The model under review builds one solid part; all positions refer to its coordinate system, in mm. A direction names the side the tool comes from. Round coordinates to 2 decimals unless told otherwise and drop trailing zeros. Loops run counter-clockwise (first coordinate to the right, second up) from the corner with the lowest first, then second, coordinate; pieces in that order, holes last. Notation, with made-up numbers: M 52,11.25 L 95,11.25 A15 ccw 95,24.25 Z; hole C 25.25,64.5 d3. An arc over 180 degrees is marked long. One line per question, with ' | ' between items.
from build123d import *

# Parameters (mm, degrees)
SKETCH1_W                                          = 80
SKETCH1_H                                          = 100
BOSS_EXTRUDE1_DEPTH                                = 120
SKETCH2_R                                          = 20
CUT_EXTRUDE1_DEPTH                                 = 137.014705087
HOLE_SIZE_BASED_ON_HEX_SOCKET_CAP_SCRE_D           = 10
HOLE_SIZE_BASED_ON_HEX_SOCKET_CAP_SCRE_DEPTH       = 35
HOLE_SIZE_BASED_ON_HEX_SOCKET_CAP_SCRE_CBORE_D     = 15
HOLE_SIZE_BASED_ON_HEX_SOCKET_CAP_SCRE_CBORE_DEPTH = 9
HOLE_SIZE_BASED_ON_HEX_SOCKET_CAP_SCRE_TIP         = 3.004303095
HOLE_WIZARD_2_D                                    = 10
HOLE_WIZARD_2_DEPTH                                = 50
HOLE_WIZARD_2_CBORE_D                              = 15
HOLE_WIZARD_2_CBORE_DEPTH                          = 9
HOLE_WIZARD_2_TIP                                  = 3.004303095
M8_TAPPED_HOLE1_D                                  = 6.8
M8_TAPPED_HOLE1_DEPTH                              = 30
M8_TAPPED_HOLE1_TIP                                = 2.042926105
M8_TAPPED_HOLE2_D                                  = 6.8
M8_TAPPED_HOLE2_DEPTH                              = 30
M8_TAPPED_HOLE2_TIP                                = 2.042926105
M8_TAPPED_HOLE3_D                                  = 6.8
M8_TAPPED_HOLE3_DEPTH                              = 45
M8_TAPPED_HOLE3_TIP                                = 2.042926105


with BuildPart() as part:
    # Sketch1 → Boss-Extrude1 (new body)
    with BuildSketch(Plane.XY):
        Rectangle(SKETCH1_W, SKETCH1_H)
    extrude(amount=BOSS_EXTRUDE1_DEPTH)

    # Sketch2 → Cut-Extrude1 (cut, through all)
    with BuildSketch(Plane.XY.offset(120)):
        Circle(SKETCH2_R)
    extrude(amount=-CUT_EXTRUDE1_DEPTH, mode=Mode.SUBTRACT)

    # Hole Size (based on) hex socket cap screw type 2
    with Locations(Plane(origin=(0, 50, 0), x_dir=(1, 0, 0), z_dir=(0, 1, 0))):
        with Locations((0, -20), (0, -100)):
            CounterBoreHole(HOLE_SIZE_BASED_ON_HEX_SOCKET_CAP_SCRE_D / 2, HOLE_SIZE_BASED_ON_HEX_SOCKET_CAP_SCRE_CBORE_D / 2, HOLE_SIZE_BASED_ON_HEX_SOCKET_CAP_SCRE_CBORE_DEPTH, depth=HOLE_SIZE_BASED_ON_HEX_SOCKET_CAP_SCRE_DEPTH)
            with Locations((0, 0, -(HOLE_SIZE_BASED_ON_HEX_SOCKET_CAP_SCRE_DEPTH + HOLE_SIZE_BASED_ON_HEX_SOCKET_CAP_SCRE_TIP / 2))):  # 118° drill point
                Cone(0, HOLE_SIZE_BASED_ON_HEX_SOCKET_CAP_SCRE_D / 2, HOLE_SIZE_BASED_ON_HEX_SOCKET_CAP_SCRE_TIP, mode=Mode.SUBTRACT)

    # 打孔尺寸(%根据)内六角圆柱头螺钉的类型2
    with Locations(Plane(origin=(0, -50, 0), x_dir=(-1, 0, 0), z_dir=(0, -1, 0))):
        with Locations((0, -20), (0, -100)):
            CounterBoreHole(HOLE_WIZARD_2_D / 2, HOLE_WIZARD_2_CBORE_D / 2, HOLE_WIZARD_2_CBORE_DEPTH, depth=HOLE_WIZARD_2_DEPTH)
            with Locations((0, 0, -(HOLE_WIZARD_2_DEPTH + HOLE_WIZARD_2_TIP / 2))):  # 118° drill point
                Cone(0, HOLE_WIZARD_2_D / 2, HOLE_WIZARD_2_TIP, mode=Mode.SUBTRACT)

    # M8 Tapped Hole1
    with Locations(Plane.ZY.offset(40)):
        with Locations((30, 30), (90, 30), (90, -30), (30, -30)):
            Hole(M8_TAPPED_HOLE1_D / 2, depth=M8_TAPPED_HOLE1_DEPTH)
            with Locations((0, 0, -(M8_TAPPED_HOLE1_DEPTH + M8_TAPPED_HOLE1_TIP / 2))):  # 118° drill point
                Cone(0, M8_TAPPED_HOLE1_D / 2, M8_TAPPED_HOLE1_TIP, mode=Mode.SUBTRACT)

    # M8 Tapped Hole2
    with Locations(Plane(origin=(40, 0, 0), x_dir=(0, 0, -1), z_dir=(1, 0, 0))):
        with Locations((-90, 30), (-30, 30), (-30, -30), (-90, -30)):
            Hole(M8_TAPPED_HOLE2_D / 2, depth=M8_TAPPED_HOLE2_DEPTH)
            with Locations((0, 0, -(M8_TAPPED_HOLE2_DEPTH + M8_TAPPED_HOLE2_TIP / 2))):  # 118° drill point
                Cone(0, M8_TAPPED_HOLE2_D / 2, M8_TAPPED_HOLE2_TIP, mode=Mode.SUBTRACT)

    # M8 Tapped Hole3
    with Locations(Plane(origin=(0, 50, 0), x_dir=(1, 0, 0), z_dir=(0, 1, 0))):
        with Locations((0, -60)):
            Hole(M8_TAPPED_HOLE3_D / 2, depth=M8_TAPPED_HOLE3_DEPTH)
            with Locations((0, 0, -(M8_TAPPED_HOLE3_DEPTH + M8_TAPPED_HOLE3_TIP / 2))):  # 118° drill point
                Cone(0, M8_TAPPED_HOLE3_D / 2, M8_TAPPED_HOLE3_TIP, mode=Mode.SUBTRACT)


solid = part.part
1) Mouldability with a two-part tool opening along Z and no side actions: class faces 1 (the flat face through (17, 12, 0)), 2 (the flat face through (5, 41, 22)), 3 (the cylindrical face through (1.08, 30.03, 24.88)), 4 (the flat face through (-40, -1, 59)) as +Z half, -Z half, draft (parallel to the pull), parting line (faces both ways), or undercut.
Output values:
face 1: -Z half | face 2: undercut | face 3: undercut | face 4: draft
2) Add section C-C on x = 16.5. State the section outline as (y, z) points, then the cut area to 3 significant figures.
Output values:
outline: M -50,0 L -11.3,0 L -11.3,120 L -50,120 Z; M 11.3,0 L 50,0 L 50,120 L 11.3,120 Z; hole C -30,30 d6.8; hole C -30,90 d6.8; hole C 30,30 d6.8; hole C 30,90 d6.8 | area: 9,140 mm²
3) Add section A-A on y = 43.5. State the section outline as (x, z) points, then the cut area to 3 significant figures.
Output values:
outline: M -40,0 L 40,0 L 40,120 L -40,120 Z; hole C 0,20 d15; hole C 0,100 d15; hole C 0,60 d6.8 | area: 9,210 mm²
4) For line 1 (Z direction, x = 0, y = -30); line 2 (Z direction, x = 0, y = 47.5); line 3 (Z direction, x = -25.75, y = -30), list the stretches that pass through material, from the lowest coordinate up.
Output values:
line 1: z = 0 to 15, 25 to 95, 105 to 120 | line 2: z = 0 to 12.5, 27.5 to 56.6, 63.4 to 92.5, 107.5 to 120 | line 3: z = 0 to 26.6, 33.4 to 86.6, 93.4 to 120
5) Add section B-B on z = 20. State the section outline as (x, y) points, then the cut area to 3 significant figures.
Output values:
outline: M -40,-50 L -7.5,-50 L -7.5,-41 L -5,-41 L -5,-19.36 A20 cw -5,19.36 L -5,41 L -7.5,41 L -7.5,50 L -40,50 Z; M 5,-41 L 7.5,-41 L 7.5,-50 L 40,-50 L 40,50 L 7.5,50 L 7.5,41 L 5,41 L 5,19.36 A20 cw 5,-19.36 Z | area: 6,050 mm²
6) Add section D-D on z = 70.5. State the section outline as (x, y) points, then the cut area to 3 significant figures.
Output values:
outline: M -40,-50 L 40,-50 L 40,50 L -40,50 Z; hole C 0,0 d40 | area: 6,740 mm²
7) Machinability: for faces 5 (the cylindrical face through (1.63, -45.56, 107.32)), 6 (the cylindrical face through (0.74, 34.64, 63.32)), 7 (the cylindrical face through (-24.79, 27.931, 92.698)), 8 (the cylindrical face through (24.8, -29.9, 86.6)), which of the approach directions +Z, -Z, +X, -X, +Y, -Y give a long, thin tool a straight path to every point of the face, cutting with its end or side? Answer none if there is none.
Output values:
face 5: -Y | face 6: +Y | face 7: -X | face 8: +X
8) Insertion check: P1, Ø4.5, axis at x = -2.5, z = 20.5, coming from the -Y side; P2, Ø8, axis at y = 30, z = 30, coming from the -X side; P3, Ø11.5, axis at x = 0, z = 100, coming from the -Y side; P4, Ø6, axis at y = -30, z = 30, coming from the +X side. Each pin has a flat end and moves straight along its axis. Give the tip position at first contact, or say it passes through.
Output values:
P1: passes through | P2: stops at x = -40 | P3: stops at y = -41 | P4: stops at x = 9.76
